```python
from build123d import *

# Parameters (mm, degrees)
SKETCH_1_W                  = 1283
SKETCH_1_H                  = 1093
EXTRUDE_1_DEPTH             = 1.5
FILLET_1_R                  = 5
HOLE_WIZARD_6_5_6_5_1_D     = 6.5
HOLE_WIZARD_6_5_6_5_1_DEPTH = 15.61
HOLE_WIZARD_6_5_6_5_1_TIP   = 1.876388375
SKETCH_5_R                  = 15
CUT_EXTRUDE_1_DEPTH         = 10
HOLE_WIZARD_6_5_6_5_2_D     = 6.5
HOLE_WIZARD_6_5_6_5_2_DEPTH = 15.61
HOLE_WIZARD_6_5_6_5_2_TIP   = 1.876388375


with BuildPart() as part:
    # 草图1 → 凸台-拉伸1 (new body)
    with BuildSketch(Plane.XY):
        Rectangle(SKETCH_1_W, SKETCH_1_H)
    extrude(amount=EXTRUDE_1_DEPTH)

    # 圆角1
    fillet_1_edges = [part.edges().sort_by_distance(p)[0] for p in [
        (-641.5, 546.5, 0.75),
        (641.5, 546.5, 0.75),
        (641.5, -546.5, 0.75),
        (-641.5, -546.5, 0.75),
    ]]
    fillet(fillet_1_edges, radius=FILLET_1_R)

    # Ø6.5 (6.5) 直径孔1
    with Locations(Plane.XY.offset(1.5)):
        with Locations((0, 526.5), (400, 526.5), (-400, 526.5), (-621.5, 300), (-621.5, 0), (-621.5, -300), (-400, -526.5), (0, -526.5), (400, -526.5), (621.5, 300), (621.5, 0), (621.5, -300), (-621.5, 526.5), (-621.5, -526.5), (621.5, -526.5), (621.5, 526.5)):
            Hole(HOLE_WIZARD_6_5_6_5_1_D / 2, depth=HOLE_WIZARD_6_5_6_5_1_DEPTH)
            with Locations((0, 0, -(HOLE_WIZARD_6_5_6_5_1_DEPTH + HOLE_WIZARD_6_5_6_5_1_TIP / 2))):  # 120° drill point
                Cone(0, HOLE_WIZARD_6_5_6_5_1_D / 2, HOLE_WIZARD_6_5_6_5_1_TIP, mode=Mode.SUBTRACT)

    # 草图5 → 切除-拉伸1 (cut)
    with BuildSketch(Plane.XY.offset(1.5)):
        with Locations((-541.5, -446.5)):
            Circle(SKETCH_5_R)
    extrude(amount=-CUT_EXTRUDE_1_DEPTH, mode=Mode.SUBTRACT)

    # Ø6.5 (6.5) 直径孔2
    with Locations(Plane.XY.offset(1.5)):
        with Locations((-561.284609691, -433.5), (-540.5, -469.5), (-519.715390309, -433.5)):
            Hole(HOLE_WIZARD_6_5_6_5_2_D / 2, depth=HOLE_WIZARD_6_5_6_5_2_DEPTH)
            with Locations((0, 0, -(HOLE_WIZARD_6_5_6_5_2_DEPTH + HOLE_WIZARD_6_5_6_5_2_TIP / 2))):  # 120° drill point
                Cone(0, HOLE_WIZARD_6_5_6_5_2_D / 2, HOLE_WIZARD_6_5_6_5_2_TIP, mode=Mode.SUBTRACT)


solid = part.part
```
Work out the finished part from the listing and answer in its coordinate system (mm). Give positions to 0.01 mm unless a question says otherwise; leave off trailing zeros. Write item = value, one per line.
Q1. A flat-ended cylindrical pin translates along its axis: pin 1 Ø4 at (x, y) = (-621.5, 0) entering from +Z. Find the tip coordinate at first contact, or state that the pin passes through.
Computed values:
pin_1 = through
Q2. Consider line 1 along X through (y, z) = (-300, 1); line 2 along Y through (x, z) = (-541.5, 0.75); line 3 along Y through (x, z) = (-621.5, 0.3). Determine where each line is inside the solid, lowest interval first.
Computed values:
line_1 = -641.5 to -624.75, -618.25 to 618.25, 624.75 to 641.5
line_2 = -546.5 to -472.59, -466.41 to -461.5, -431.5 to 546.5
line_3 = -546.5 to -529.75, -523.25 to -303.25, -296.75 to -3.25, 3.25 to 296.75, 303.25 to 523.25, 529.75 to 546.5
Q3. For a pull along Y with two mould halves and no side action, classify faces 1 (the cylindrical face through (-533.44, -433.85, 0.76)), 2 (the flat face through (-9, 8, 1.5)) as pulls with the +Y half, pulls with the -Y half, needs draft (parallel to the pull), parting line crosses it, or undercut.
Computed values:
face_1 = undercut
face_2 = needs draft
